Read the model definition and answer for the solid it produces. Units are mm, in the model's axes. Face numbers are marked on the shaded views. A direction names the side the tool comes from. Coordinates: 2 decimals unless noted, no trailing zeros. Write each loop counter-clockwise with the first axis right and the second up, starting at its lowest first coordinate (ties: lowest second). Pieces come first, ordered by that corner, then holes.
(1) Which of the six approach directions +Z, -Z, +X, -X, +Y, -Y give full straight-line access (tool end or side, diameter ignored) to the marked faces 1, 2, 3 and 4?
(2) The mould has two halves that part along X. Classify the marked faces 5, 6, 7 and 8: +X half, -X half, draft (parallel to the pull), parting line (faces both ways), or undercut.
(3) Given pin 1 (7.5 mm diameter, centred on y = 12.5, z = 11, fed in from -X); pin 2 (8 mm diameter, centred on x = -0.5, z = -5, fed in from +Y); pin 3 (5 mm diameter, centred on x = -40.5, y = -15, fed in from +Z), each flat-ended and moving along its own axis, determine where each tip first touches the part or whether it passes through.
(4) Section A-A on x = 12 is taken. Write down the section's boundary in (y, z).
(5) Section B-B on y = -12 is taken. Write down the section's boundary in (x, z).
(6) Section D-D on x = 37 is taken. Write down the section's boundary in (y, z).
(7) Find the intervals of material crossed by probe 1 along Y at (x, z) = (-59.5, 10); probe 2 along X at (y, z) = (3, 15); probe 3 along Z at (x, y) = (-46.5, -15.5), in increasing order.
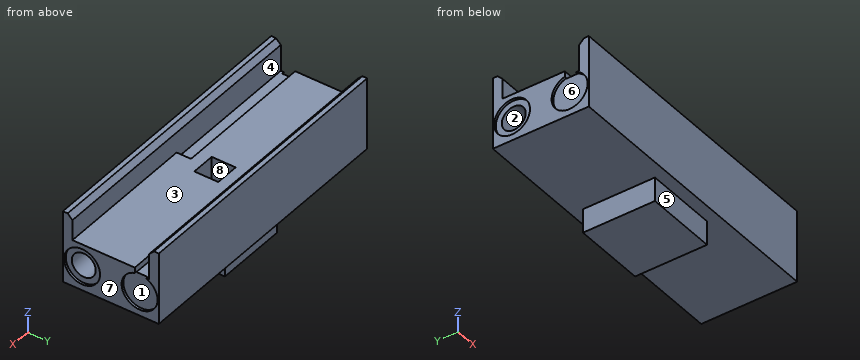
from build123d import *

# Parameters (mm, degrees)
SKETCH1_W           = 120
SKETCH1_H           = 40
BOSS_EXTRUDE1_DEPTH = 30
CUT_EXTRUDE1_DEPTH  = 70
CUT_EXTRUDE2_DEPTH  = 60
SKETCH5_W           = 30
SKETCH5_H           = 30
BOSS_EXTRUDE2_DEPTH = 10
SKETCH7_W           = 10
SKETCH7_H           = 10
CUT_EXTRUDE4_DEPTH  = 10
CHAMFER1_SIZE       = 2
SKETCH6_R           = 7.5
CUT_EXTRUDE5_DEPTH  = 1
SKETCH9_R           = 5
CUT_EXTRUDE6_DEPTH  = 55
SKETCH10_R          = 5
CUT_EXTRUDE7_DEPTH  = 55


with BuildPart() as part:
    # Sketch1 → Boss-Extrude1 (new body)
    with BuildSketch(Plane.XY):
        Rectangle(SKETCH1_W, SKETCH1_H)
    extrude(amount=BOSS_EXTRUDE1_DEPTH)

    # Sketch3 → Cut-Extrude1 (cut)
    with BuildSketch(Plane(origin=(60, 0, 0), x_dir=(0, 0, -1), z_dir=(1, 0, 0))):
        Polygon((-30, 16), (-17, 16), (-17, 10), (-19.5, 10), (-19.5, -16), (-30, -16), align=None)
    extrude(amount=-CUT_EXTRUDE1_DEPTH, mode=Mode.SUBTRACT)

    # Sketch4 → Cut-Extrude2 (cut)
    with BuildSketch(Plane.ZY.offset(60)):
        Polygon((30, 16), (19.5, 16), (19.5, -10), (17, -10), (17, -16), (30, -16), align=None)
    extrude(amount=-CUT_EXTRUDE2_DEPTH, mode=Mode.SUBTRACT)

    # Sketch5 → Boss-Extrude2 (add)
    with BuildSketch(Plane(origin=(0, 0, 0), x_dir=(-1, 0, 0), z_dir=(0, 0, -1))):
        Rectangle(SKETCH5_W, SKETCH5_H)
    extrude(amount=BOSS_EXTRUDE2_DEPTH)

    # Sketch7 → Cut-Extrude4 (cut)
    with BuildSketch(Plane.XY.offset(19.5)):
        Rectangle(SKETCH7_W, SKETCH7_H)
    extrude(amount=-CUT_EXTRUDE4_DEPTH, mode=Mode.SUBTRACT)

    # Chamfer1
    chamfer1_edges = [part.edges().sort_by_distance(p)[0] for p in [
        (0, -16, 30),
        (0, 16, 30),
    ]]
    chamfer(chamfer1_edges, length=CHAMFER1_SIZE)

    # Sketch6 → Cut-Extrude5 (cut)
    with BuildSketch(Plane(origin=(60, 0, 0), x_dir=(0, 0, -1), z_dir=(1, 0, 0))):
        with Locations((-10, 12)):
            Circle(SKETCH6_R)
        with Locations(Location((-10, -12, 0), (0, 0, 90))):
            Circle(SKETCH6_R)
    cut_extrude5 = extrude(amount=-CUT_EXTRUDE5_DEPTH, mode=Mode.SUBTRACT)

    # Sketch9 → Cut-Extrude6 (cut)
    with BuildSketch(Plane(origin=(59, 0, 0), x_dir=(0, 0, -1), z_dir=(1, 0, 0))):
        with Locations(Location((-10, -12, 0), (0, 0, 90))):
            Circle(SKETCH9_R)
    extrude(amount=-CUT_EXTRUDE6_DEPTH, mode=Mode.SUBTRACT)

    # Mirror1: Cut-Extrude5 across plane
    add(cut_extrude5.mirror(Plane(origin=(0, 0, 0), x_dir=(0, 0, 1), z_dir=(1, 0, 0))), mode=Mode.SUBTRACT)

    # Sketch10 → Cut-Extrude7 (cut)
    with BuildSketch(Plane.ZY.offset(59)):
        with Locations(Location((10, 12, 0), (0, 0, 270))):
            Circle(SKETCH10_R)
    extrude(amount=-CUT_EXTRUDE7_DEPTH, mode=Mode.SUBTRACT)


solid = part.part
Response:
1. face 1: +X
1. face 2: -X
1. face 3: +Z, +X, -X
1. face 4: +Z, -X
2. face 5: draft
2. face 6: -X half
2. face 7: +X half
2. face 8: undercut
3. pin 1: stops at x = -4
3. pin 2: stops at y = 15
3. pin 3: stops at z = 29.5
4. outline: (-20, 0) - (-15, 0) - (-15, -10) - (15, -10) - (15, 0) - (20, 0) - (20, 30) - (18, 30) - (16, 28) - (16, 17) - (10, 17) - (10, 19.5) - (-16, 19.5) - (-16, 28) - (-18, 30) - (-20, 30) - close; hole circle Ø10 at (-12, 10)
5. outline: (-60, 0) - (-15, 0) - (-15, -10) - (15, -10) - (15, 0) - (60, 0) - (60, 2.5) - (59, 2.5) - (59, 5) - (4, 5) - (4, 15) - (59, 15) - (59, 17.5) - (60, 17.5) - (60, 19.5) - (0, 19.5) - (0, 17) - (-59, 17) - (-59, 2.5) - (-60, 2.5) - close
6. outline: (-20, 0) - (20, 0) - (20, 30) - (18, 30) - (16, 28) - (16, 17) - (10, 17) - (10, 19.5) - (-16, 19.5) - (-16, 28) - (-18, 30) - (-20, 30) - close; hole circle Ø10 at (-12, 10)
7. probe 1: y = -20 to -19.5, -4.5 to 4.5, 19.5 to 20
7. probe 2: x = -60 to -5, 5 to 60
7. probe 3: z = 0 to 17
